Design review of the part shown in the three views and the two pictorial views. Dimensions are in mm from the part's minimum x, y and z. Coordinates: 2 decimals unless noted, no trailing zeros. Loops run counter-clockwise (first coordinate to the right, second up) from the corner with the lowest first, then second, coordinate; pieces in that order, holes last. Notation, with made-up numbers: (78, -9.5) -> (116, -9.5) arc R16 cw to (116, 8.5) -> close; hole circle Ø1 at (59.25, 14.5). An arc over 180 degrees is marked (long way). Answer in a Markdown table with one row per item.
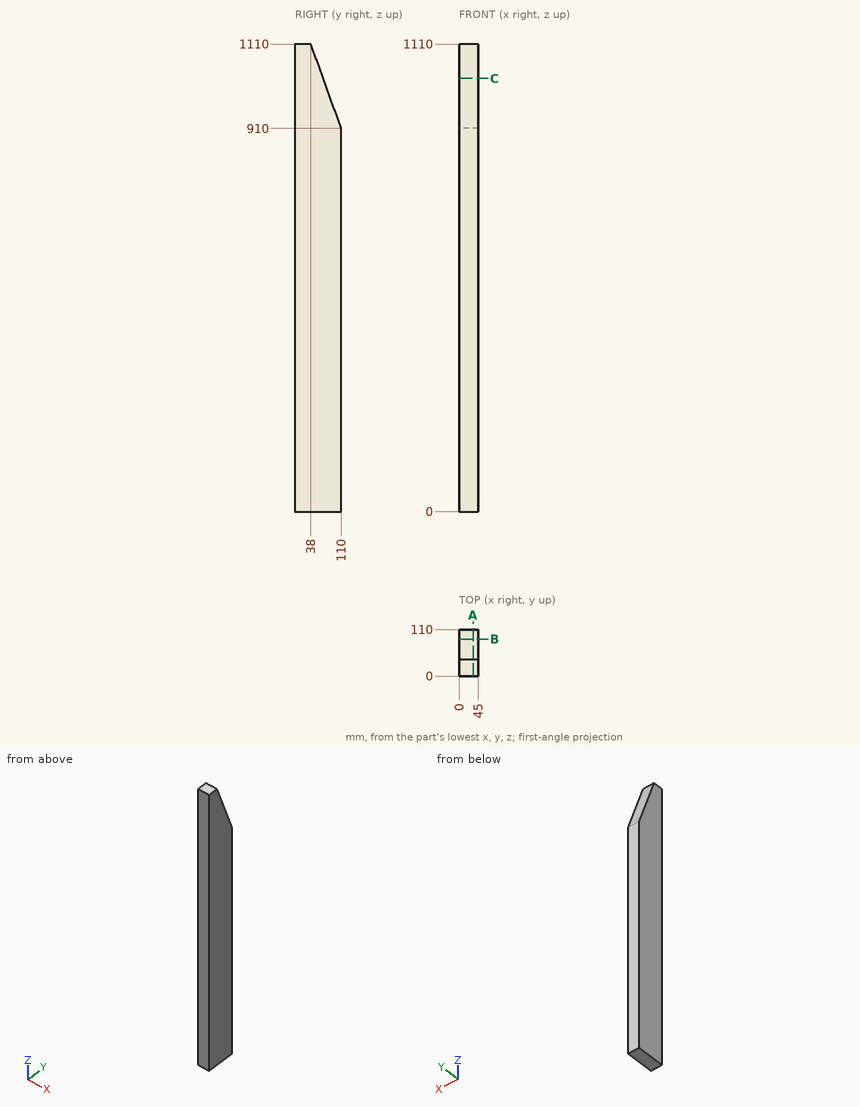
Item 1: Take a section at C-C, the plane z = 1028.5. State the section outline as (x, y) points, and give its area (3 significant figures).
Worked answers:
| item | result |
|---|---|
| outline | (0, 0) -> (45, 0) -> (45, 67.34) -> (0, 67.34) -> close |
| area | 3,030 mm² |
Item 2: For L1, parallel to Y at x = 5, z = 992.5; L2, parallel to Y at x = 33, z = 1065, list the stretches that pass through material, from the lowest coordinate up.
Worked answers:
| item | result |
|---|---|
| L1 | 0 to 80.3 |
| L2 | 0 to 54.2 |
Item 3: Take a section at A-A, the plane x = 33. State the section outline as (y, z) points, and give its area (3 significant figures).
Worked answers:
| item | result |
|---|---|
| outline | (0, 0) -> (110, 0) -> (110, 910) -> (38, 1110) -> (0, 1110) -> close |
| area | 115,000 mm² |
Item 4: Take a section at B-B, the plane y = 87.5. State the section outline as (x, z) points, and give its area (3 significant figures).
Worked answers:
| item | result |
|---|---|
| outline | (0, 0) -> (45, 0) -> (45, 972.5) -> (0, 972.5) -> close |
| area | 43,800 mm² |
